Work out the finished part from the listing and answer in its coordinate system (mm). A direction names the side the tool comes from. Give positions to 0.01 mm unless a question says otherwise; leave off trailing zeros. Loops run counter-clockwise (first coordinate to the right, second up) from the corner with the lowest first, then second, coordinate; pieces in that order, holes last. Notation, with made-up numbers: M 49,23.25 L 67,23.25 A12 cw 67,32.25 Z; hole C 7.25,-9.5 d8. An arc over 180 degrees is marked long. Answer in a Markdown table with one row per item. Add a question column.
from build123d import *

# Parameters (mm, degrees)
SKETCH1_W                      = 80
SKETCH1_H                      = 199.7
BOSS_EXTRUDE1_DEPTH            = 80
F_8_5_8_5_DIAMETER_HOLE1_D     = 8.5
F_8_5_8_5_DIAMETER_HOLE1_DEPTH = 20
F_8_5_8_5_DIAMETER_HOLE1_TIP   = 2.553657631
FILLET2_R                      = 10
SKETCH5_R                      = 13
CUT_EXTRUDE1_DEPTH             = 100
F_8_5_8_5_DIAMETER_HOLE2_D     = 8.5
F_8_5_8_5_DIAMETER_HOLE2_DEPTH = 20
F_8_5_8_5_DIAMETER_HOLE2_TIP   = 2.553657631


with BuildPart() as part:
    # Sketch1 → Boss-Extrude1 (new body)
    with BuildSketch(Plane(origin=(0, 0, -30), x_dir=(-1, 0, 0), z_dir=(0, 0, -1))):
        with Locations((0, 99.85)):
            Rectangle(SKETCH1_W, SKETCH1_H)
    extrude(amount=-BOSS_EXTRUDE1_DEPTH)

    # Ø8.5 (8.5) Diameter Hole1
    with Locations(Plane(origin=(40, 0, 0), x_dir=(0, 0, -1), z_dir=(1, 0, 0))):
        with Locations((-10, 30), (-10, 179.7), (-10, 70)):
            Hole(F_8_5_8_5_DIAMETER_HOLE1_D / 2, depth=F_8_5_8_5_DIAMETER_HOLE1_DEPTH)
            with Locations((0, 0, -(F_8_5_8_5_DIAMETER_HOLE1_DEPTH + F_8_5_8_5_DIAMETER_HOLE1_TIP / 2))):  # 118° drill point
                Cone(0, F_8_5_8_5_DIAMETER_HOLE1_D / 2, F_8_5_8_5_DIAMETER_HOLE1_TIP, mode=Mode.SUBTRACT)

    # Fillet2
    fillet2_edges = [part.edges().sort_by_distance(p)[0] for p in [
        (-40, 99.85, 50),
        (40, 99.85, 50),
        (-40, 99.85, -30),
        (40, 99.85, -30),
    ]]
    fillet(fillet2_edges, radius=FILLET2_R)

    # Sketch5 → Cut-Extrude1 (cut)
    with BuildSketch(Plane.XZ):
        with Locations((0, 10)):
            Circle(SKETCH5_R)
    extrude(amount=-CUT_EXTRUDE1_DEPTH, mode=Mode.SUBTRACT)

    # Ø8.5 (8.5) Diameter Hole2
    with Locations(Plane(origin=(40, 0, 0), x_dir=(0, 0, -1), z_dir=(1, 0, 0))):
        with Locations((-10, 139.7)):
            Hole(F_8_5_8_5_DIAMETER_HOLE2_D / 2, depth=F_8_5_8_5_DIAMETER_HOLE2_DEPTH)
            with Locations((0, 0, -(F_8_5_8_5_DIAMETER_HOLE2_DEPTH + F_8_5_8_5_DIAMETER_HOLE2_TIP / 2))):  # 118° drill point
                Cone(0, F_8_5_8_5_DIAMETER_HOLE2_D / 2, F_8_5_8_5_DIAMETER_HOLE2_TIP, mode=Mode.SUBTRACT)


solid = part.part
(1) Section A-A, the plane y = 61.5 is taken. Determine the outline of the cut face in (x, z), and give its area (3 significant figures).
(2) Which of the six approach directions +Z, -Z, +X, -X, +Y, -Y give full straight-line access (tool end or side, diameter ignored) to faces 1 (the face through (0, 100, 10)), 2 (the face through (1, 199.7, 9)), 3 (the face through (29.86, 143.914, 9.447))?
(3) Section D-D, the plane x = -33.5 is taken. Determine the outline of the cut face in (y, z), and give its area (3 significant figures).
(4) Consider line 1 along Y through (x, z) = (27.5, 10); line 2 along Z through (x, y) = (24, 179.7); line 3 along Z through (x, y) = (0, 62). Determine where each line is inside the solid, lowest interval first. Write a range as from..to.
(5) This flat-tipped pin is pushed along its axis until it touches: P1, Ø8, axis at x = 4.5, z = 4, coming from the -Y side. Where does it stop, or does it pass through?
(6) Section C-C, the plane z = 2 is taken. Determine the outline of the cut face in (x, y), and give its area (3 significant figures).
(7) Section B-B, the plane x = 0 is taken. Determine the outline of the cut face in (y, z), and give its area (3 significant figures).
(8) The mould has two halves that part along Z. Classify faces 4 (the face through (0, 101, 50)), 5 (the face through (17.89, 138.98, 10.16)), 6 (the face through (-40, 98, 10)): pulls with the +Z half, pulls with the -Z half, needs draft (parallel to the pull), parting line crosses it, or undercut.
Numbers:
| question | item | result |
|---|---|---|
| 1 | outline | M -40,-20 A10 ccw -30,-30 L 30,-30 A10 ccw 40,-20 L 40,40 A10 ccw 30,50 L -30,50 A10 ccw -40,40 Z; hole C 0,10 d26 |
| 1 | area | 5,780 mm² |
| 2 | face 1 | -Y |
| 2 | face 2 | +Z, -Z, +X, -X, +Y |
| 2 | face 3 | +X |
| 3 | outline | M 0,-29.37 L 199.7,-29.37 L 199.7,49.37 L 0,49.37 Z |
| 3 | area | 15,700 mm² |
| 4 | line 1 | y = 0..25.75, 34.25..65.75, 74.25..135.45, 143.95..175.45, 183.95..199.7 |
| 4 | line 2 | z = -30..5.75, 14.25..50 |
| 4 | line 3 | z = -30..-3, 23..50 |
| 5 | P1 | stops at y = 100 |
| 6 | outline | M -40,0 L -10.25,0 L -10.25,100 L 10.25,100 L 10.25,0 L 40,0 L 40,199.7 L -40,199.7 Z |
| 6 | area | 13,900 mm² |
| 7 | outline | M 0,-30 L 199.7,-30 L 199.7,50 L 0,50 L 0,23 L 100,23 L 100,-3 L 0,-3 Z |
| 7 | area | 13,400 mm² |
| 8 | face 4 | pulls with the +Z half |
| 8 | face 5 | undercut |
| 8 | face 6 | needs draft |
